from build123d import *

# Parameters (mm, degrees)
SKETCH1_W           = 60
SKETCH1_H           = 55
SKETCH1_R           = 8.5
BOSS_EXTRUDE1_DEPTH = 12
CHAMFER1_SIZE       = 10


with BuildPart() as part:
    # Sketch1 → Boss-Extrude1 (new body)
    with BuildSketch(Plane(origin=(0, 0, 0), x_dir=(1, 0, 0), z_dir=(0, 1, 0))):
        with Locations((30, -27.5)):
            Rectangle(SKETCH1_W, SKETCH1_H)
        with Locations(Location((30, -30, 0), (0, 0, 270))):
            Circle(SKETCH1_R, mode=Mode.SUBTRACT)
    extrude(amount=BOSS_EXTRUDE1_DEPTH)

    # Chamfer1
    chamfer1_edges = [part.edges().sort_by_distance(p)[0] for p in [
        (60, 6, 55),
        (0, 6, 55),
    ]]
    chamfer(chamfer1_edges, length=CHAMFER1_SIZE)


solid = part.part
CAD build for the part. Positions are in the model's coordinates, mm. Give positions to 0.01 mm unless a question says otherwise; leave off trailing zeros. Loops run counter-clockwise (first coordinate to the right, second up) from the corner with the lowest first, then second, coordinate; pieces in that order, holes last. Notation, with made-up numbers: M 66,21 L 78,21 A32 ccw 78,48 Z; hole C -33,28.25 d2. An arc over 180 degrees is marked long. Answer in a Markdown table with one row per item. Add a question column.
Item 1: Band-saw the part on B-B on z = 30. Give the cut face in (x, y), then the cut area to 3 significant figures.
Item 2: Band-saw the part on A-A on x = 30. Give the cut face in (y, z).
Item 3: Band-saw the part on D-D on z = 46. Give the cut face in (x, y), then the cut area to 3 significant figures.
Item 4: Mould opens along X. For faces 1 (the face through (30, 0, 21)), 2 (the face through (60, 6, 23)), 3 (the face through (22.46, 5.92, 33.92)) say: +X half, -X half, draft (parallel to the pull), parting line (faces both ways), or undercut.
Item 5: Drop a flat-ended pin along its axis: P1, Ø10, axis at x = 30, z = 30, coming from the -Y side. Give the stop position or say it passes through.
Item 6: Probe probe 1 along X at (y, z) = (9.25, 30); probe 2 along X at (y, z) = (0.5, 23.5); probe 3 along Z at (x, y) = (53, 8.5). List the from-to ranges inside material, lowest first.
Item 7: Band-saw the part on C-C on y = 10.75. Give the cut face in (x, z), then the cut area to 3 significant figures.
Reply:
| question | item | result |
|---|---|---|
| 1 | outline | M 0,0 L 21.5,0 L 21.5,12 L 0,12 Z; M 38.5,0 L 60,0 L 60,12 L 38.5,12 Z |
| 1 | area | 516 mm^2 |
| 2 | outline | M 0,0 L 12,0 L 12,21.5 L 0,21.5 Z; M 0,38.5 L 12,38.5 L 12,55 L 0,55 Z |
| 3 | outline | M 1,0 L 59,0 L 59,12 L 1,12 Z |
| 3 | area | 696 mm^2 |
| 4 | face 1 | draft |
| 4 | face 2 | +X half |
| 4 | face 3 | undercut |
| 5 | P1 | passes through |
| 6 | probe 1 | x = 0 to 21.5, 38.5 to 60 |
| 6 | probe 2 | x = 0 to 24.52, 35.48 to 60 |
| 6 | probe 3 | z = 0 to 52 |
| 7 | outline | M 0,0 L 60,0 L 60,45 L 50,55 L 10,55 L 0,45 Z; hole C 30,30 d17 |
| 7 | area | 2,970 mm^2 |
